Source: three-view drawing plus pictorial views. Frame: mm from the lowest corner of the part. A direction names the side the tool comes from. Give positions to 0.01 mm unless a question says otherwise; leave off trailing zeros. Loops run counter-clockwise (first coordinate to the right, second up) from the corner with the lowest first, then second, coordinate; pieces in that order, holes last. Notation, with made-up numbers: (-18, 0.25) - (19, 0.25) arc R21 ccw to (19, 11.25) - close; hole circle Ø9 at (-10, 33.5). An arc over 180 degrees is marked (long way). Answer as a JSON object with one key per item and string values.
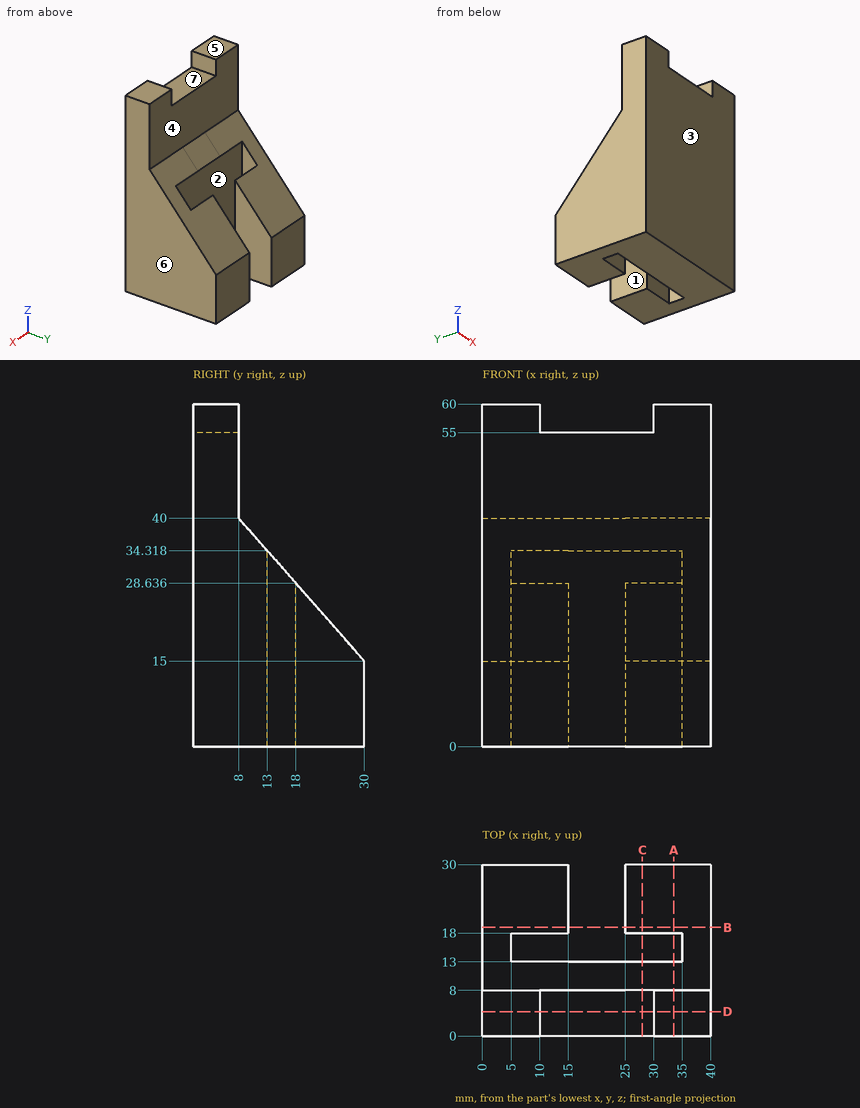
Item 1: Mould query, pull axis X, two halves, no side actions, for the marked faces 5, 6 and 7. Classes: released by +X, released by -X, zero draft, split by the parting line, or undercut.
Geometry check:
{"face 5": "zero draft", "face 6": "released by +X", "face 7": "undercut"}
Item 2: Material intervals for line 1 (X direction, y = 23.5, z = 8); line 2 (X direction, y = 15.5, z = 30); line 3 (Y direction, x = 22.5, z = 34), sorted ascending. Write a range as [from, to].
Geometry check:
{"line 1": "x = [0, 15], [25, 40]", "line 2": "x = [0, 5], [35, 40]", "line 3": "y = [0, 13]"}
Item 3: Cut plane A-A (x = 33.5). Return loops of the section in (y, z).
Geometry check:
{"outline": "(0, 0) - (13, 0) - (13, 34.32) - (8, 40) - (8, 60) - (0, 60) - close; (18, 0) - (30, 0) - (30, 15) - (18, 28.64) - close"}
Item 4: Cut plane D-D (y = 4.25). Return loops of the section in (x, z).
Geometry check:
{"outline": "(0, 0) - (40, 0) - (40, 60) - (30, 60) - (30, 55) - (10, 55) - (10, 60) - (0, 60) - close"}
Item 5: Access query for the marked faces 1, 2, 3 and 4. Directions: +Z, -Z, +X, -X, +Y, -Y. A direction counts if a zero-diameter tool reaches every point of the face in a straight line with its end or side. Return the directions, or none.
Geometry check:
{"face 1": "+Z, -Z, +Y", "face 2": "+Z, -Z", "face 3": "+Z, -Z, +X, -X, -Y", "face 4": "+Z, +X, -X, +Y"}
Item 6: Cut plane C-C (x = 28). Return loops of the section in (y, z).
Geometry check:
{"outline": "(0, 0) - (13, 0) - (13, 34.32) - (8, 40) - (8, 55) - (0, 55) - close; (18, 0) - (30, 0) - (30, 15) - (18, 28.64) - close"}
Item 7: Cut plane B-B (y = 19). Return loops of the section in (x, z), then the cut area to 3 significant figures.
Geometry check:
{"outline": "(0, 0) - (15, 0) - (15, 27.5) - (0, 27.5) - close; (25, 0) - (40, 0) - (40, 27.5) - (25, 27.5) - close", "area": "825 mm2"}
Item 8: Contact query for flat-ended pins moving along their axis: P1, Ø4, axis at x = 19, y = 5.5, coming from the +Z side; P2, Ø6, axis at x = 22.5, z = 24, coming from the +Y side; P3, Ø12, axis at x = 27.5, z = 34, coming from the +Y side. Output: stop coordinate, or through.
Geometry check:
{"P1": "stops at z = 55", "P2": "stops at y = 23.54", "P3": "stops at y = 18.56"}
